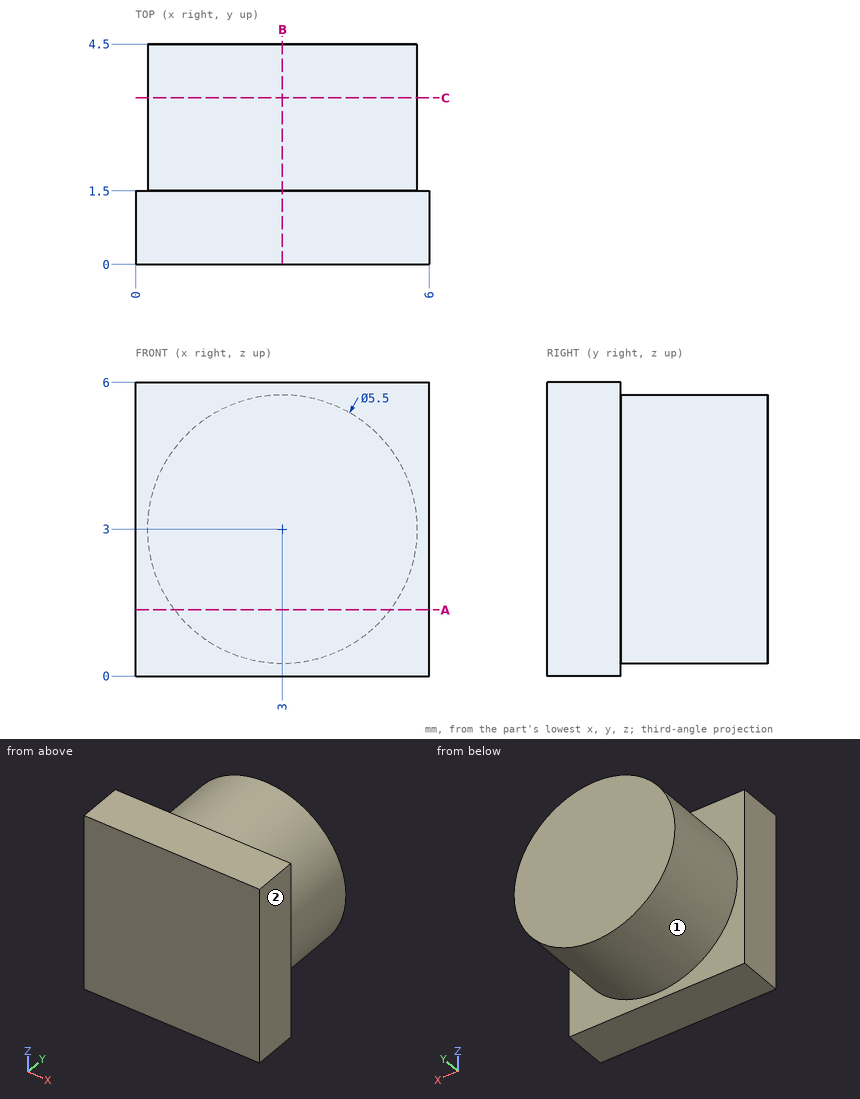
Verification items for this drawing (mm, ordinates from the low corner). A direction names the side the tool comes from. Coordinates: 2 decimals unless noted, no trailing zeros. Write each loop counter-clockwise with the first axis right and the second up, starting at its lowest first coordinate (ties: lowest second). Pieces come first, ordered by that corner, then holes. Notation, with made-up numbers: M -23.75,87 L 26.25,87 A23 cw 26.25,111 Z; hole C 9,-36.5 d7. An arc over 180 degrees is marked long. Use one line per item in the form item = value. Start each with the question number.
1) Section check C-C on y = 3.4. Enter the section's corners in (x, z).
2) Section check A-A on z = 1.35. Enter the section's corners in (x, y), and give its area (3 significant figures).
3) Go/stop test with a flat-tipped pin: pin 1 Ø1 at (y, z) = (2.5, 3.5) entering from -X. Record where the tip stops, or that it passes through.
4) Thickness scan on probe 1 along Y at (x, z) = (1.6, 5.4); probe 2 along X at (y, z) = (3.5, 3.05); probe 3 along X at (y, z) = (3.5, 5.5). Record the ranges inside material, lowest first. Write a range as from..to.
5) Section check B-B on x = 3. Enter the section's corners in (y, z).
6) Set-up check for the marked faces 1 and 2: record each of +Z, -Z, +X, -X, +Y, -Y from which the full face is reachable in a straight line by a thin tool's end or side.
Responses:
q1.outline = C 3,3 d5.5
q2.outline = M 0,0 L 6,0 L 6,1.5 L 5.2,1.5 L 5.2,4.5 L 0.8,4.5 L 0.8,1.5 L 0,1.5 Z
q2.area = 22.2 mm2
q3.pin_1 = 0.25
q4.probe_1 = 0..1.5
q4.probe_2 = 0.25..5.75
q4.probe_3 = 1.85..4.15
q5.outline = M 0,0 L 1.5,0 L 1.5,0.25 L 4.5,0.25 L 4.5,5.75 L 1.5,5.75 L 1.5,6 L 0,6 Z
q6.face_1 = +Y
q6.face_2 = +Z, -Z, +X, +Y, -Y
